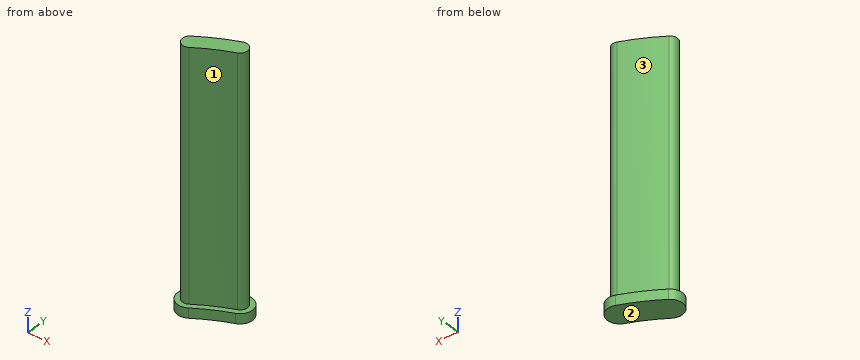
from build123d import *

# Parameters (mm, degrees)
BOSS_EXTRUDE1_DEPTH      = 20
BOSS_EXTRUDE1_DEPTH_BACK = 230
BOSS_EXTRUDE2_DEPTH      = 10


with BuildPart() as part:
    # Sketch1 → Boss-Extrude1 (new, two sides: drawn at the far end of the back side and taken through both)
    with BuildSketch(Plane.XY.offset(-BOSS_EXTRUDE1_DEPTH_BACK)):
        with BuildLine():
            ThreePointArc((-367.185078684, 365.188666312), (-385.937282785, 356.235559249), (-403.644999576, 345.361735137))
            ThreePointArc((-403.644999576, 345.361735137), (-405.565426886, 334.930438049), (-395.134129798, 333.010010739))
            ThreePointArc((-395.134129798, 333.010010739), (-378.77130289, 343.057974791), (-361.443316822, 351.33109904))
            ThreePointArc((-361.443316822, 351.33109904), (-357.385414117, 361.130763607), (-367.185078684, 365.188666312))
        make_face()
    extrude(amount=BOSS_EXTRUDE1_DEPTH + BOSS_EXTRUDE1_DEPTH_BACK)

    # Sketch2 → Boss-Extrude2 (add)
    with BuildSketch(Plane(origin=(0, 0, -230), x_dir=(-1, 0, 0), z_dir=(0, 0, -1))):
        with BuildLine():
            ThreePointArc((406.481956169, 349.478976603), (388.32594275, 360.628087401), (369.098999305, 369.807855403))
            ThreePointArc((369.098999305, 369.807855403), (352.766225026, 363.044684228), (359.529396201, 346.711909949))
            ThreePointArc((359.529396201, 346.711909949), (376.382642925, 338.665446638), (392.297173205, 328.892769272))
            ThreePointArc((392.297173205, 328.892769272), (409.682668352, 332.093481456), (406.481956169, 349.478976603))
        make_face()
    extrude(amount=BOSS_EXTRUDE2_DEPTH)


solid = part.part
Geometry: final body of the model. Coordinates: model frame, mm. Face numbers are marked on the shaded views. A direction names the side the tool comes from. Give positions to 0.01 mm unless a question says otherwise; leave off trailing zeros. Write each loop counter-clockwise with the first axis right and the second up, starting at its lowest first coordinate (ties: lowest second). Pieces come first, ordered by that corner, then holes.
(1) First-contact query: P1, Ø10, axis at y = 360, z = -61, coming from the +X side; P2, Ø8, axis at x = -384, z = -56, coming from the -Y side; P3, Ø2, axis at x = -386.5, z = -191, coming from the -Y side. Flat tips, straight axial feed; report the tip coordinate or a pass-through.
(2) Cut plane C-C, the plane z = -52. Return loops of the section in (x, y) (3 decimals), then the cut area to 3 significant figures.
(3) Access query for the marked faces 1, 2 and 3. Directions: +Z, -Z, +X, -X, +Y, -Y. A direction counts if a zero-diameter tool reaches every point of the face in a straight line with its end or side. Return the directions, or none.
(4) Cut plane B-B, the plane x = -382. Return loops of the section in (y, z), then the cut area to 3 significant figures.
(5) Cut plane A-A, the plane y = 342.5. Return loops of the section in (x, z).
(6) Ray query, line 1 (X direction, y = 333, z = -135); line 2 (Z direction, x = -404, y = 348); line 3 (Y direction, x = -361.5, z = -188.5). Return the intervals inside material, ascending.
Values follow:
1. P1: stops at x = -356.81
1. P2: stops at y = 337.68
1. P3: stops at y = 337.99
2. outline: (-403.645, 345.362) arc R7.5 ccw to (-395.134, 333.01) arc R182.5 cw to (-361.443, 351.331) arc R7.5 ccw to (-367.185, 365.189) arc R197.5 ccw to start
2. area: 777 mm2
3. face 1: +Z, +X, -Y
3. face 2: -Z, +X, -X, +Y, -Y
3. face 3: +Z, -X, +Y
4. outline: (335.48, -240) - (363.93, -240) - (363.93, -230) - (358.32, -230) - (358.32, 20) - (341.26, 20) - (341.26, -230) - (335.48, -230) - close
4. area: 4,550 mm2
5. outline: (-411.44, -240) - (-368.92, -240) - (-368.92, -230) - (-379.79, -230) - (-379.79, 20) - (-406.12, 20) - (-406.12, -230) - (-411.44, -230) - close
6. line 1: x = -403.63 to -395.15
6. line 2: z = -240 to -230
6. line 3: y = 351.31 to 365.21
